```python
from build123d import *

# Parameters (mm, degrees)
SKETCH_1_R          = 5.0528125
EXTRUDE_597_DEPTH   = 10.8
SKETCH_2_OUTSIDE_W  = 89.934
SKETCH_2_OUTSIDE_H  = 92.718
SKETCH_2_OUTSIDE_R  = 9
CUT_EXTRUDE_1_DEPTH = 18.482562741
CUT_EXTRUDE_1_DRAFT = -60
SKETCH_3_OUTSIDE_W  = 89.934
SKETCH_3_OUTSIDE_H  = 92.718
SKETCH_3_OUTSIDE_R  = 9
CUT_EXTRUDE_2_DEPTH = 18.482562741
CUT_EXTRUDE_2_DRAFT = -60


with BuildPart() as part:
    # 草图1 → Extrude 597 (new body)
    with BuildSketch(Plane.XY):
        Polygon((0, 10.392304845), (-9, 5.196152423), (-9, -5.196152423), (0, -10.392304845), (9, -5.196152423), (9, 5.196152423), align=None)
        with Locations(Location((0, 0, 0), (0, 0, 180))):
            Circle(SKETCH_1_R, mode=Mode.SUBTRACT)
    extrude(amount=EXTRUDE_597_DEPTH)


with BuildPart() as cut_extrude_1_tool:
    # 草图2 outside → 切除-拉伸1 (with draft: the straight prism first)
    with BuildSketch(Plane(origin=(0, 0, 0), x_dir=(-1, 0, 0), z_dir=(0, 0, -1))):
        Rectangle(SKETCH_2_OUTSIDE_W, SKETCH_2_OUTSIDE_H)
        Circle(SKETCH_2_OUTSIDE_R, mode=Mode.SUBTRACT)
    extrude(amount=-CUT_EXTRUDE_1_DEPTH)
    # 切除-拉伸1: the draft: its side faces are tilted about the plane it starts from
    cut_extrude_1_sides = [cut_extrude_1_tool.faces().sort_by_distance(p)[0] for p in [
        (0, -46.359, 9.241281371),
        (-44.967, 0, 9.241281371),
        (0, 46.359, 9.241281371),
        (44.967, 0, 9.241281371),
        (9, 0, 9.241281371),
    ]]
    draft(cut_extrude_1_sides, Plane(origin=(0, 0, 0), x_dir=(-1, 0, 0), z_dir=(0, 0, -1)), CUT_EXTRUDE_1_DRAFT)


with BuildPart() as part_1:
    add(part.part)

    # 切除-拉伸1: cut by cut_extrude_1_tool
    add(cut_extrude_1_tool.part, mode=Mode.SUBTRACT)


with BuildPart() as cut_extrude_2_tool:
    # 草图3 outside → 切除-拉伸2 (with draft: the straight prism first)
    with BuildSketch(Plane.XY.offset(10.8)):
        Rectangle(SKETCH_3_OUTSIDE_W, SKETCH_3_OUTSIDE_H)
        Circle(SKETCH_3_OUTSIDE_R, mode=Mode.SUBTRACT)
    extrude(amount=-CUT_EXTRUDE_2_DEPTH)
    # 切除-拉伸2: the draft: its side faces are tilted about the plane it starts from
    cut_extrude_2_sides = [cut_extrude_2_tool.faces().sort_by_distance(p)[0] for p in [
        (0, -46.359, 1.558718629),
        (44.967, 0, 1.558718629),
        (0, 46.359, 1.558718629),
        (-44.967, 0, 1.558718629),
        (-9, 0, 1.558718629),
    ]]
    draft(cut_extrude_2_sides, Plane.XY.offset(10.8), CUT_EXTRUDE_2_DRAFT)


with BuildPart() as part_2:
    add(part_1.part)

    # 切除-拉伸2: cut by cut_extrude_2_tool
    add(cut_extrude_2_tool.part, mode=Mode.SUBTRACT)


solid = part_2.part
```
Geometry check sheet. Reference: the model listing, model coordinates, mm. Round coordinates to 2 decimals unless told otherwise and drop trailing zeros. Order: outer loops, then holes, each group sorted by start corner. A loop starts at its lowest first (then second) coordinate and runs counter-clockwise, first axis right, second up. Notation, with made-up numbers: (19, 22.5) -> (76, 22.5) arc R14 cw to (76, 27.5) -> close; hole circle Ø4 at (82, 70). An arc over 180 degrees is marked (long way). Return JSON: item names as keys, results as strings. Group by question number.
Q1. Release check for a two-part mould opening along X. For faces 1 (the cylindrical face through (-4.82, -1.52, 5.32)), 2 (the flat face through (9, 0, 5)), 3 (the flat face through (-4.56, -7.76, 5.32)), 4 (the conical face through (-0.02, -9.33, 10.61)) record: released by +X, released by -X, zero draft, split by the parting line, or undercut.
Q2. Material ranges on probe 1 along Y at (x, z) = (-3.25, 7); probe 2 along Y at (x, z) = (0, 10.5); probe 3 along X at (y, z) = (0.5, 8.75), recorded low to high. Write a range as from..to.
Q3. Gauge pin test, flat ends, axial feed: pin 1 (3 mm diameter, centred on y = -8, z = 8.5, fed in from -X); pin 2 (1 mm diameter, centred on x = 5, z = 5, fed in from -Y). Record the tip position at first contact, or that the pin passes through.
Q4. Section check A-A, the plane z = 1.25. Record the boundary of the cut face in (x, y), plus the area to 3 significant figures.
Q5. Section check B-B, the plane z = 10.25. Record the boundary of the cut face in (x, y).
Numbers:
{
 "1": {"face 1": "undercut", "face 2": "released by +X", "face 3": "released by -X", "face 4": "split by the parting line"},
 "2": {"probe 1": "-8.52..-3.87, 3.87..8.52", "probe 2": "-9.52..-5.05, 5.05..9.52", "probe 3": "-9..-5.03, 5.03..9"},
 "3": {"pin 1": "x = -6.74", "pin 2": "y = -7.79"},
 "4": {"outline": "(-9, -5.2) -> (0, -10.39) -> (9, -5.2) -> (9, 5.2) -> (0, 10.39) -> (-9, 5.2) -> close; hole circle Ø10.11 at (0, 0)", "area": "200 mm^2"},
 "5": {"outline": "(-9, -4.25) arc R9.95 ccw to (-8.18, -5.67) -> (-0.82, -9.92) arc R9.95 ccw to (0.82, -9.92) -> (8.18, -5.67) arc R9.95 ccw to (9, -4.25) -> (9, 4.25) arc R9.95 ccw to (8.18, 5.67) -> (0.82, 9.92) arc R9.95 ccw to (-0.82, 9.92) -> (-8.18, 5.67) arc R9.95 ccw to (-9, 4.25) -> close; hole circle Ø10.11 at (0, 0)"}
}
